Check sheet for the modelled part. Datum: model origin and axes. Units: mm. Face numbers are marked on the shaded views. A direction names the side the tool comes from. Round coordinates to 2 decimals unless told otherwise and drop trailing zeros. Order: outer loops, then holes, each group sorted by start corner. A loop starts at its lowest first (then second) coordinate and runs counter-clockwise, first axis right, second up. Notation, with made-up numbers: (23.5, 86) -> (59.5, 86) arc R17 cw to (59.5, 97) -> close; hole circle Ø2 at (-23.75, 60.5). An arc over 180 degrees is marked (long way). Answer in a Markdown table with one row per item.
from build123d import *

# Parameters (mm, degrees)
BASE_PLATE_DEPTH        = 20
HEX_MOUNTING_BOSS_DEPTH = 50
GUSSET_RIB_1_SKETCH_W   = 8
GUSSET_RIB_1_SKETCH_H   = 40
GUSSET_RIB_1_DEPTH      = 16
RIB_1_TRIM_CUT_DEPTH    = 16
GUSSET_RIB_2_SKETCH_W   = 8
GUSSET_RIB_2_SKETCH_H   = 40
GUSSET_RIB_2_DEPTH      = 16
RIB_2_TRIM_CUT_DEPTH    = 16
BOSS_BORE_20_D          = 20
BOSS_BORE_20_DEPTH      = 55
BOSS_BORE_20_TIP        = 6.00860619
SHAFT_HOUSING_DEPTH     = 36
HOUSING_FILLET_R10_R    = 10
HOUSING_POCKET_DEPTH    = 31
HOUSING_SLOT_DEPTH      = 13
CROSS_HOLE_6_D          = 6
CROSS_HOLE_6_DEPTH      = 20
CROSS_HOLE_6_TIP        = 1.802581857


with BuildPart() as part:
    # Base Plate Sketch → Base Plate (new body)
    with BuildSketch(Plane(origin=(0, 0, 0), x_dir=(1, 0, 0), z_dir=(0, 1, 0))):
        with BuildLine():
            Line((0, 40), (106, 40))
            Line((106, 40), (112, 34))
            Line((112, 34), (112, -34))
            Line((112, -34), (106, -40))
            Line((106, -40), (0, -40))
            ThreePointArc((0, -40), (-40, 0), (0, 40))
        make_face()
    extrude(amount=BASE_PLATE_DEPTH)

    # Hex Boss Sketch → Hex Mounting Boss (add)
    with BuildSketch(Plane(origin=(0, 20, 0), x_dir=(1, 0, 0), z_dir=(0, 1, 0))):
        Polygon((0, 24.248711306), (-21, 12.124355653), (-21, -12.124355653), (0, -24.248711306), (21, -12.124355653), (21, 12.124355653), align=None)
    extrude(amount=HEX_MOUNTING_BOSS_DEPTH)

    # Gusset Rib 1 Sketch → Gusset Rib 1 (add)
    with BuildSketch(Plane(origin=(-10.5, 0, 18.186533479), x_dir=(0.8660254037844417, 0, 0.4999999999999949), z_dir=(-0.4999999999999949, 0, 0.8660254037844417))):
        with Locations((0, 40)):
            Rectangle(GUSSET_RIB_1_SKETCH_W, GUSSET_RIB_1_SKETCH_H)
    extrude(amount=GUSSET_RIB_1_DEPTH)

    # Rib 1 Trim Sketch → Rib 1 Trim Cut (cut)
    with BuildSketch(Plane(origin=(3.464101615, 0, 2), x_dir=(0.49999999999999495, 0, -0.8660254037844417), z_dir=(0.8660254037844417, 0, 0.49999999999999495))):
        Polygon((-21, 60), (-37, 20), (-37, 60), align=None)
    extrude(amount=-RIB_1_TRIM_CUT_DEPTH, mode=Mode.SUBTRACT)

    # Gusset Rib 2 Sketch → Gusset Rib 2 (add)
    with BuildSketch(Plane(origin=(-10.5, 0, -18.186533479), x_dir=(-0.8660254037844386, 0, 0.4999999999999999), z_dir=(-0.49999999999999994, 0, -0.8660254037844387))):
        with Locations((0, 40)):
            Rectangle(GUSSET_RIB_2_SKETCH_W, GUSSET_RIB_2_SKETCH_H)
    extrude(amount=GUSSET_RIB_2_DEPTH)

    # Rib 2 Trim Sketch → Rib 2 Trim Cut (cut)
    with BuildSketch(Plane(origin=(-3.464101615, 0, 2), x_dir=(0.5000000000000001, 0, 0.8660254037844386), z_dir=(-0.8660254037844386, 0, 0.5000000000000001))):
        Polygon((-21, 60), (-37, 20), (-37, 60), align=None)
    extrude(amount=-RIB_2_TRIM_CUT_DEPTH, mode=Mode.SUBTRACT)

    # Boss Bore Ø20
    with Locations(Plane(origin=(0, 70, 0), x_dir=(1, 0, 0), z_dir=(0, 1, 0))):
        with Locations((0, 0)):
            Hole(BOSS_BORE_20_D / 2, depth=BOSS_BORE_20_DEPTH)
            with Locations((0, 0, -(BOSS_BORE_20_DEPTH + BOSS_BORE_20_TIP / 2))):  # 118° drill point
                Cone(0, BOSS_BORE_20_D / 2, BOSS_BORE_20_TIP, mode=Mode.SUBTRACT)

    # Shaft Housing Sketch → Shaft Housing (add)
    with BuildSketch(Plane(origin=(0, 20, 0), x_dir=(1, 0, 0), z_dir=(0, 1, 0))):
        Polygon((112, 25), (62, 25), (62, 5), (21, 5), (21, -5), (62, -5), (62, -25), (112, -25), align=None)
    extrude(amount=SHAFT_HOUSING_DEPTH)

    # Housing Fillet R10
    housing_fillet_r10_edges = [part.edges().sort_by_distance(p)[0] for p in [
        (62, 38, -25),
        (62, 38, 25),
    ]]
    fillet(housing_fillet_r10_edges, radius=HOUSING_FILLET_R10_R)

    # Housing Pocket Sketch → Housing Pocket (cut)
    with BuildSketch(Plane(origin=(0, 56, 0), x_dir=(1, 0, 0), z_dir=(0, 1, 0))):
        with BuildLine():
            Line((112, 17.5), (73, 17.5))
            ThreePointArc((73, 17.5), (69.464466094, 16.035533906), (68, 12.5))
            Line((68, 12.5), (68, -12.5))
            ThreePointArc((68, -12.5), (69.464466094, -16.035533906), (73, -17.5))
            Line((73, -17.5), (112, -17.5))
            Line((112, -17.5), (112, 17.5))
        make_face()
    extrude(amount=-HOUSING_POCKET_DEPTH, mode=Mode.SUBTRACT)

    # Housing Slot Sketch → Housing Slot (cut)
    with BuildSketch(Plane(origin=(0, 25, 0), x_dir=(1, 0, 0), z_dir=(0, 1, 0))):
        with BuildLine():
            Line((86, 10), (112, 10))
            Line((112, 10), (112, -10))
            Line((112, -10), (86, -10))
            ThreePointArc((86, -10), (76, 0), (86, 10))
        make_face()
    extrude(amount=-HOUSING_SLOT_DEPTH, mode=Mode.SUBTRACT)

    # Cross Hole Ø6
    with Locations(Plane(origin=(0, 56, 0), x_dir=(1, 0, 0), z_dir=(0, 1, 0))):
        with Locations((40, 0)):
            Hole(CROSS_HOLE_6_D / 2, depth=CROSS_HOLE_6_DEPTH)
            with Locations((0, 0, -(CROSS_HOLE_6_DEPTH + CROSS_HOLE_6_TIP / 2))):  # 118° drill point
                Cone(0, CROSS_HOLE_6_D / 2, CROSS_HOLE_6_TIP, mode=Mode.SUBTRACT)


solid = part.part
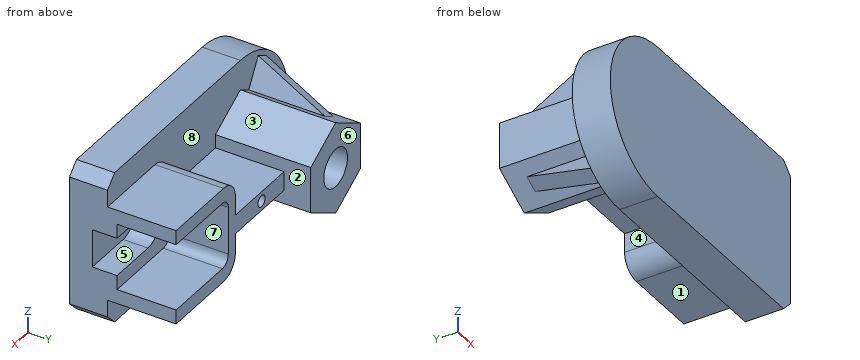
Item 1: Mould release check, pull along X, two halves, no side actions. Record for the marked faces 6, 7 and 8: pulls with the +X half, pulls with the -X half, needs draft (parallel to the pull), parting line crosses it, or undercut.
Result sheet:
| item | result |
|---|---|
| face 6 | needs draft |
| face 7 | pulls with the +X half |
| face 8 | undercut |
Item 2: Cross-section at A-A (x = 44.5). Record the boundary of the cut face in (y, z), and give its area (3 significant figures).
Result sheet:
| item | result |
|---|---|
| outline | (0, -40) -> (20, -40) -> (20, -5) -> (56, -5) -> (56, 5) -> (20, 5) -> (20, 40) -> (0, 40) -> close |
| area | 1,960 mm^2 |
Item 3: Depth check by flat-ended pin: P1, Ø15.5, axis at x = 90, y = 36, coming from the +Z side; P2, Ø1.5, axis at y = 28, z = 22.5, coming from the -X side; P3, Ø25, axis at x = 96, y = 37.5, coming from the -Z side; P4, Ø1.5, axis at y = 40, z = 28.5, coming from the +X side. Enter the tip coordinate at first touch or a pass-through.
Result sheet:
| item | result |
|---|---|
| P1 | stops at z = 25 |
| P2 | stops at x = -18.04 |
| P3 | stops at z = -25 |
| P4 | passes through |
Item 4: Scan lines: line 1 (Z direction, x = 40, y = 49); line 2 (Z direction, x = -15.5, y = 30.5); line 3 (Z direction, x = 0, y = 50). Record each from-to range of solid material in increasing order. Write a range as [from, to].
Result sheet:
| item | result |
|---|---|
| line 1 | z = [-5, -3], [3, 5] |
| line 2 | z = [-28.93, -18.85], [-15.3, 15.3], [18.85, 28.93] |
| line 3 | z = [-24.25, -10], [10, 24.25] |
Item 5: Cross-section at C-C (z = -26.5). Record the boundary of the cut face in (x, y), and give its area (3 significant figures).
Result sheet:
| item | result |
|---|---|
| outline | (-29.96, 0) -> (112, 0) -> (112, 20) -> (-10.68, 20) -> (-10.68, 41.77) -> (-19.92, 30.23) -> (-19.92, 20) -> (-29.96, 20) -> close |
| area | 2,990 mm^2 |
Item 6: Set-up check for the marked faces 1, 2, 3, 4 and 5: record each of +Z, -Z, +X, -X, +Y, -Y from which the full face is reachable in a straight line by a thin tool's end or side.
Result sheet:
| item | result |
|---|---|
| face 1 | -Z, +X, +Y |
| face 2 | +Y |
| face 3 | +Z, +Y |
| face 4 | -Z, +Y |
| face 5 | +X, +Y |
Item 7: Cross-section at B-B (y = 49.5). State how many separate pieces and enclosed holes the cut face has, and give its area (3 significant figures).
Result sheet:
| item | result |
|---|---|
| separate pieces | 1 |
| enclosed holes | 2 |
| area | 2,590 mm^2 |
